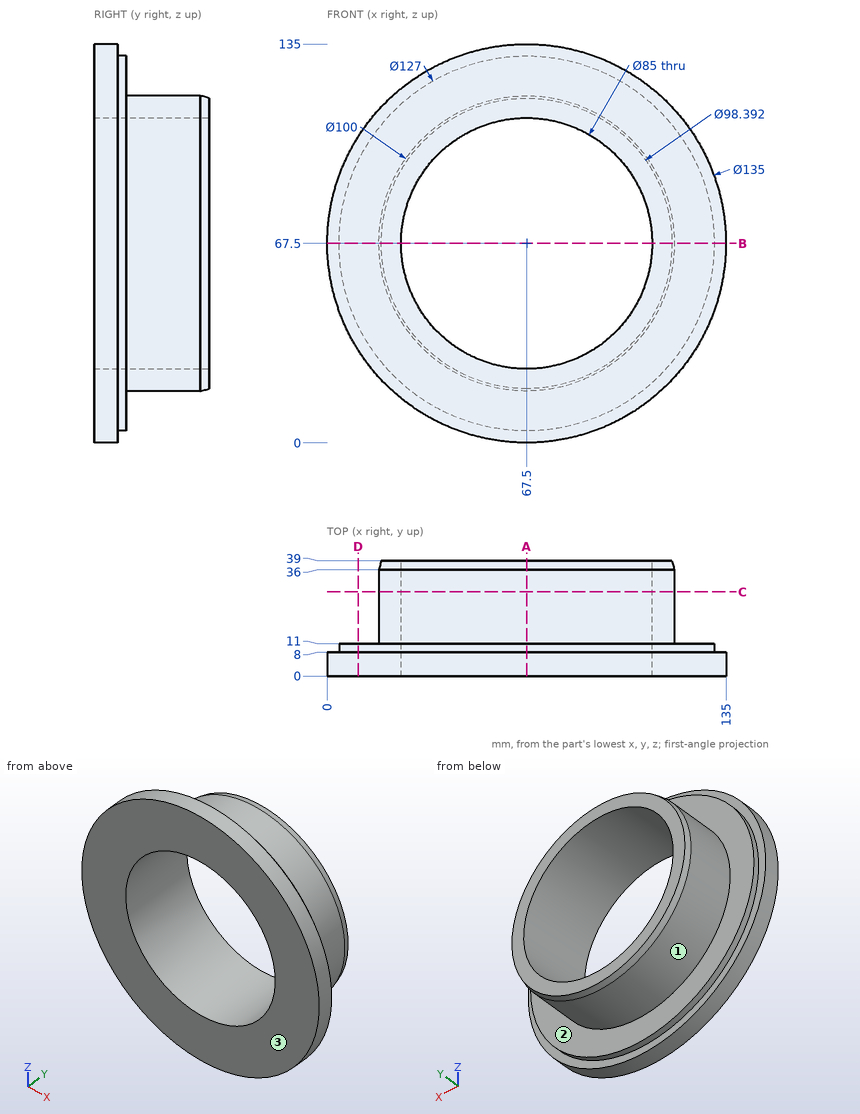
Check sheet for the drawn part. Datum: minimum x, y, z corner. Units: mm. Give positions to 0.01 mm unless a question says otherwise; leave off trailing zeros. Order: outer loops, then holes, each group sorted by start corner. A loop starts at its lowest first (then second) coordinate and runs counter-clockwise, first axis right, second up. Notation, with made-up numbers: (-11.5, 11.5) -> (45.5, 11.5) arc R26 cw to (45.5, 38.5) -> close; hole circle Ø9 at (-15.75, -19.5). An arc over 180 degrees is marked (long way). Answer as CSV lines item,"result".
Q1. Scan lines: probe 1 along X at (y, z) = (26, 67.5); probe 2 along Y at (x, z) = (13, 32). Record each from-to range of solid material in increasing order.
Solutions:
probe 1,"x = 17.5 to 25, 110 to 117.5"
probe 2,"y = 0 to 8"
Q2. Sectioned sample at D-D on x = 10.5. Record the cut outline in (y, z).
Solutions:
outline,"(0, 31.34) -> (8, 31.34) -> (8, 39.51) -> (11, 39.51) -> (11, 95.49) -> (8, 95.49) -> (8, 103.66) -> (0, 103.66) -> close"
Q3. Sectioned sample at A-A on x = 67.5. Record the cut outline in (y, z).
Solutions:
outline,"(0, 0) -> (8, 0) -> (8, 4) -> (11, 4) -> (11, 17.5) -> (36, 17.5) -> (39, 18.3) -> (39, 25) -> (0, 25) -> close; (0, 110) -> (39, 110) -> (39, 116.7) -> (36, 117.5) -> (11, 117.5) -> (11, 131) -> (8, 131) -> (8, 135) -> (0, 135) -> close"
Q4. Release check for a two-part mould opening along Y. For the marked faces 1, 2 and 3 record: +Y half, -Y half, draft (parallel to the pull), parting line (faces both ways), or undercut.
Solutions:
face 1,"draft"
face 2,"+Y half"
face 3,"-Y half"
Q5. Depth check by flat-ended pin: pin 1 (1 mm diameter, centred on y = 24, z = 34.5, fed in from +X); pin 2 (4 mm diameter, centred on y = 31, z = 60.5, fed in from +X); pin 3 (12 mm diameter, centred on x = 26.5, y = 4.5, fed in from +Z). Enter the tip coordinate at first touch or a pass-through.
Solutions:
pin 1,"stops at x = 105.5"
pin 2,"stops at x = 117.25"
pin 3,"stops at z = 125.22"
Q6. Sectioned sample at B-B on z = 67.5. Record the cut outline in (x, y).
Solutions:
outline,"(0, 0) -> (25, 0) -> (25, 39) -> (18.3, 39) -> (17.5, 36) -> (17.5, 11) -> (4, 11) -> (4, 8) -> (0, 8) -> close; (110, 0) -> (135, 0) -> (135, 8) -> (131, 8) -> (131, 11) -> (117.5, 11) -> (117.5, 36) -> (116.7, 39) -> (110, 39) -> close"
Q7. Sectioned sample at C-C on y = 28.5. Record the cut outline in (x, z), plus the area to 3 significant figures.
Solutions:
outline,"circle Ø100 at (67.5, 67.5); hole circle Ø85 at (67.5, 67.5)"
area,"2,180 mm²"
